Verification items for the finished model (mm, model axes). Face numbers are marked on the shaded views. A direction names the side the tool comes from. Coordinates: 2 decimals unless noted, no trailing zeros. Order: outer loops, then holes, each group sorted by start corner. A loop starts at its lowest first (then second) coordinate and runs counter-clockwise, first axis right, second up. Notation, with made-up numbers: M -27,78.5 L -18,78.5 A27 ccw -18,101.5 Z; hole C 54,-2.5 d9. An arc over 180 degrees is marked long. Write item = value, one per line.
```python
from build123d import *

# Parameters (mm, degrees)
EXTRUDE_1_DEPTH     = 90
CUT_EXTRUDE_1_REACH = 97.021
CUT_EXTRUDE_2_REACH = 97.021


with BuildPart() as part:
    # 草图1 → 凸台-拉伸1 (new, symmetric)
    with BuildSketch(Plane.XY):
        Polygon((0, 0), (0, 23), (3, 23), (3, 3), (23, 3), (23, 0), align=None)
    extrude(amount=EXTRUDE_1_DEPTH, both=True)

    # 草图3 → 切除-拉伸1 (cut, up to next)
    with BuildSketch(Plane(origin=(3, 0, 0), x_dir=(0, 0, -1), z_dir=(1, 0, 0)), mode=Mode.PRIVATE) as cut_extrude_1_sk1:
        with BuildLine():
            Line((-82, 16.5), (-47, 16.5))
            ThreePointArc((-47, 16.5), (-44.5, 14), (-47, 11.5))
            Line((-47, 11.5), (-82, 11.5))
            ThreePointArc((-82, 11.5), (-84.5, 14), (-82, 16.5))
        make_face()
    cut_extrude_1_tool1 = extrude(cut_extrude_1_sk1.sketch, amount=-CUT_EXTRUDE_1_REACH, mode=Mode.PRIVATE) & part.part
    cut_extrude_1 = cut_extrude_1_tool1.solids().sort_by_distance((3, 14, 64.5))[0]
    add(cut_extrude_1, mode=Mode.SUBTRACT)

    # 镜向1: 切除-拉伸1 across plane
    add(cut_extrude_1.mirror(Plane.XY), mode=Mode.SUBTRACT)

    # 草图4 → 切除-拉伸2 (cut, up to next)
    with BuildSketch(Plane(origin=(0, 3, 0), x_dir=(1, 0, 0), z_dir=(0, 1, 0)), mode=Mode.PRIVATE) as cut_extrude_2_sk1:
        with BuildLine():
            Line((8, 42.5), (18, 42.5))
            ThreePointArc((18, 42.5), (20.5, 40), (18, 37.5))
            Line((18, 37.5), (8, 37.5))
            ThreePointArc((8, 37.5), (5.5, 40), (8, 42.5))
        make_face()
    cut_extrude_2_tool1 = extrude(cut_extrude_2_sk1.sketch, amount=-CUT_EXTRUDE_2_REACH, mode=Mode.PRIVATE) & part.part
    # 草图4 → 切除-拉伸2 (cut, up to next)
    with BuildSketch(Plane(origin=(0, 3, 0), x_dir=(1, 0, 0), z_dir=(0, 1, 0)), mode=Mode.PRIVATE) as cut_extrude_2_sk2:
        with BuildLine():
            Line((8, -37.5), (18, -37.5))
            ThreePointArc((18, -37.5), (20.5, -40), (18, -42.5))
            Line((18, -42.5), (8, -42.5))
            ThreePointArc((8, -42.5), (5.5, -40), (8, -37.5))
        make_face()
    cut_extrude_2_tool2 = extrude(cut_extrude_2_sk2.sketch, amount=-CUT_EXTRUDE_2_REACH, mode=Mode.PRIVATE) & part.part
    add(cut_extrude_2_tool1.solids().sort_by_distance((13, 3, -40))[0], mode=Mode.SUBTRACT)
    add(cut_extrude_2_tool2.solids().sort_by_distance((13, 3, 40))[0], mode=Mode.SUBTRACT)


solid = part.part
```
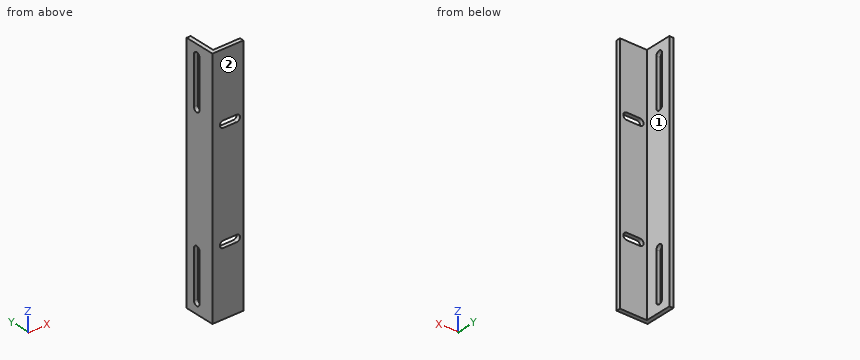
Item 1: Sectioned sample at C-C, the plane z = 33. Enter the section's corners in (x, y).
Report:
outline = M 0,0 L 23,0 L 23,3 L 3,3 L 3,23 L 0,23 Z
Item 2: Sectioned sample at B-B, the plane z = -40. Enter the section's corners in (x, y), then the cut area to 3 significant figures.
Report:
outline = M 0,0 L 5.5,0 L 5.5,3 L 3,3 L 3,23 L 0,23 Z; M 20.5,0 L 23,0 L 23,3 L 20.5,3 Z
area = 84.0 mm^2
Item 3: Sectioned sample at D-D, the plane y = 7.75. Enter the section's corners in (x, z), then the cut area to 3 significant figures.
Report:
outline = M 0,-90 L 3,-90 L 3,90 L 0,90 Z
area = 540 mm^2
Item 4: Scan lines: L1, parallel to Y at x = 2.75, z = -64; L2, parallel to Z at x = 19, y = 1.25; L3, parallel to Y at x = 21.5, z = 47. Record each from-to range of solid material in increasing order. Write a range as from..to.
Report:
L1 = 0..11.5, 16.5..23
L2 = -90..-42.29, -37.71..37.71, 42.29..90
L3 = 0..3
Item 5: Tool access check on the marked faces 1 and 2. Record the directions out of +Z, -Z, +X, -X, +Y, -Y that give a thin tool (end or side, any length) a straight path to the whole face; none if there is none.
Report:
face_1 = +Z, -Z, +X, +Y
face_2 = +Z, -Z, +X, -X, -Y
Item 6: Sectioned sample at A-A, the plane x = 13.5. Enter the section's corners in (y, z).
Report:
outline = M 0,-90 L 3,-90 L 3,-42.5 L 0,-42.5 Z; M 0,-37.5 L 3,-37.5 L 3,37.5 L 0,37.5 Z; M 0,42.5 L 3,42.5 L 3,90 L 0,90 Z
Item 7: Gauge pin test, flat ends, axial feed: pin 1 (2 mm diameter, centred on x = 4.5, z = -15, fed in from +Y); pin 2 (2 mm diameter, centred on y = 7.5, z = -72, fed in from +X). Record the tip position at first contact, or that the pin passes through.
Report:
pin_1 = 3
pin_2 = 3
